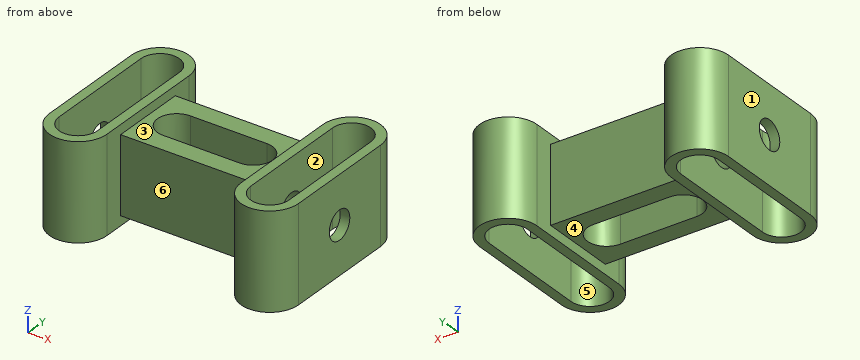
from build123d import *

# Parameters (mm, degrees)
END_PLATES_DEPTH     = 50
END_PLATES_2_DEPTH   = 50
CENTRE_WEB_PROFILE_W = 70
CENTRE_WEB_PROFILE_H = 40
CENTRE_WEB_DEPTH     = 20
CROSS_HOLE_SKETCH_R  = 7.5
CROSS_HOLE_DEPTH     = 147.372811683


with BuildPart() as part:
    # End Plates Profile → End Plates (new body)
    with BuildSketch(Plane.XY):
        with BuildLine():
            Line((15, 30), (15, -30))
            ThreePointArc((15, -30), (0, -45), (-15, -30))
            Line((-15, -30), (-15, 30))
            ThreePointArc((-15, 30), (0, 45), (15, 30))
        make_face()
        with BuildLine():
            Line((10, 30), (10, -30))
            ThreePointArc((10, -30), (0, -40), (-10, -30))
            Line((-10, -30), (-10, 30))
            ThreePointArc((-10, 30), (0, 40), (10, 30))
        make_face(mode=Mode.SUBTRACT)
    extrude(amount=END_PLATES_DEPTH)



with BuildPart() as body_2:
    # End Plates Profile → End Plates 2 (new body)
    with BuildSketch(Plane.XY):
        with BuildLine():
            Line((115, 30), (115, -30))
            ThreePointArc((115, -30), (100, -45), (85, -30))
            Line((85, -30), (85, 30))
            ThreePointArc((85, 30), (100, 45), (115, 30))
        make_face()
        with BuildLine():
            Line((110, 30), (110, -30))
            ThreePointArc((110, -30), (100, -40), (90, -30))
            Line((90, -30), (90, 30))
            ThreePointArc((90, 30), (100, 40), (110, 30))
        make_face(mode=Mode.SUBTRACT)
    extrude(amount=END_PLATES_2_DEPTH)


with BuildPart() as part_1:
    add(part.part)

    add(body_2.part)  # Centre Web merges body 2
    # Centre Web Profile → Centre Web (add, symmetric)
    with BuildSketch(Plane.XY.offset(25)):
        with Locations((50, 0)):
            Rectangle(CENTRE_WEB_PROFILE_W, CENTRE_WEB_PROFILE_H)
        with BuildLine():
            ThreePointArc((70, -10), (80, 0), (70, 10))
            Line((70, 10), (30, 10))
            ThreePointArc((30, 10), (20, 0), (30, -10))
            Line((30, -10), (70, -10))
        make_face(mode=Mode.SUBTRACT)
    extrude(amount=CENTRE_WEB_DEPTH, both=True)

    # Cross Hole Sketch → Cross Hole (cut, through all)
    with BuildSketch(Plane.ZY.offset(15)):
        with Locations(Location((25, 0, 0), (0, 0, 270))):
            Circle(CROSS_HOLE_SKETCH_R)
    extrude(amount=-CROSS_HOLE_DEPTH, mode=Mode.SUBTRACT)


solid = part_1.part
Read the model definition and answer for the solid it produces. Units are mm, in the model's axes. Face numbers are marked on the shaded views. A direction names the side the tool comes from. Round coordinates to 2 decimals unless told otherwise and drop trailing zeros. Loops run counter-clockwise (first coordinate to the right, second up) from the corner with the lowest first, then second, coordinate; pieces in that order, holes last.
Q1. Section D-D on y = 25 is taken. Write down the section's boundary in (x, z), and give its area (3 significant figures).
Q2. Which of the six approach directions +Z, -Z, +X, -X, +Y, -Y give full straight-line access (tool end or side, diameter ignored) to the marked faces 3, 4, 5 and 6?
Q3. Section C-C on y = 11.5 is taken. Write down the section's boundary in (x, z), and give its area (3 significant figures).
Q4. Each of these flat-tipped pins is pushed along its axis until it touches: pin 1 (4 mm diameter, centred on x = 84.5, y = -13, fed in from +Z); pin 2 (20 mm diameter, centred on x = 51.5, z = 26, fed in from +Y); pin 3 (8 mm diameter, centred on x = 48.5, z = 9, fed in from -Y); pin 4 (9 mm diameter, centred on y = 0, z = 25, fed in from +X). Where does it stop, or does it pass through?
Q5. Consider probe 1 along X at (y, z) = (-29, 13.5); probe 2 along X at (y, z) = (-17.5, 16.5); probe 3 along Y at (x, z) = (81.75, 25). Determine where each line is inside the solid, lowest interval first.
Q6. Section A-A on z = 38.5 is taken. Write down the section's boundary in (x, y), and give its area (3 significant figures).
Q7. Determine the mould class of the marked faces 1 and 2 for opening direction X: released by +X, released by -X, zero draft, split by the parting line, or undercut.
Q8. Section B-B on x = 0 is taken. Write down the section's boundary in (y, z), and give its area (3 significant figures).
Output:
1. outline: (-15, 0) - (-10, 0) - (-10, 50) - (-15, 50) - close; (10, 0) - (15, 0) - (15, 50) - (10, 50) - close; (85, 0) - (90, 0) - (90, 50) - (85, 50) - close; (110, 0) - (115, 0) - (115, 50) - (110, 50) - close
1. area: 1,000 mm2
2. face 3: +Z, +Y, -Y
2. face 4: -Z, +Y, -Y
2. face 5: +Z, -Z
2. face 6: +Z, -Z, -Y
3. outline: (-15, 0) - (-10, 0) - (-10, 50) - (-15, 50) - close; (10, 0) - (15, 0) - (15, 5) - (85, 5) - (85, 0) - (90, 0) - (90, 50) - (85, 50) - (85, 45) - (15, 45) - (15, 50) - (10, 50) - close; (110, 0) - (115, 0) - (115, 50) - (110, 50) - close
3. area: 3,800 mm2
4. pin 1: stops at z = 50
4. pin 2: stops at y = 20
4. pin 3: stops at y = -20
4. pin 4: passes through
5. probe 1: x = -15 to -10, 10 to 15, 85 to 90, 110 to 115
5. probe 2: x = -15 to -10, 10 to 90, 110 to 115
5. probe 3: y = -20 to -7.5, 7.5 to 20
6. outline: (-15, -30) arc R15 ccw to (15, -30) - (15, -20) - (85, -20) - (85, -30) arc R15 ccw to (115, -30) - (115, 30) arc R15 ccw to (85, 30) - (85, 20) - (15, 20) - (15, 30) arc R15 ccw to (-15, 30) - close; hole (-10, -30) arc R10 ccw to (10, -30) - (10, 30) arc R10 ccw to (-10, 30) - close; hole (30, -10) - (70, -10) arc R10 ccw to (70, 10) - (30, 10) arc R10 ccw to start; hole (90, -30) arc R10 ccw to (110, -30) - (110, 30) arc R10 ccw to (90, 30) - close
6. area: 3,670 mm2
7. face 1: released by -X
7. face 2: undercut
8. outline: (-45, 0) - (-40, 0) - (-40, 50) - (-45, 50) - close; (40, 0) - (45, 0) - (45, 50) - (40, 50) - close
8. area: 500 mm2
